Check sheet for the modelled part. Datum: model origin and axes. Units: mm. A direction names the side the tool comes from. Round coordinates to 2 decimals unless told otherwise and drop trailing zeros. Order: outer loops, then holes, each group sorted by start corner. A loop starts at its lowest first (then second) coordinate and runs counter-clockwise, first axis right, second up. Notation, with made-up numbers: M -31.75,81.5 L -11.75,81.5 A16 cw -11.75,91.5 Z; hole C 52,8.5 d8. An arc over 180 degrees is marked long. One line per item, written item: value. Start each with the question number.
(1) Release check for a two-part mould opening along X. For faces 6 (the face through (20, 123, 13)), 7 (the face through (16, 123, -9)), 8 (the face through (-13, 123, -20)) record: released by +X, released by -X, zero draft, split by the parting line, or undercut.
(2) Depth check by flat-ended pin: pin 1 Ø6 at (x, y) = (0, 161.5) entering from +Z; pin 2 Ø3.5 at (y, z) = (152, -2) entering from -X. Enter the tip coordinate at first touch or a pass-through.
(3) Access from +Z, -Z, +X, -X, +Y, -Y to the whole of each face (thin tool, end or side, straight path). Record for faces 1 (the face through (10, 123, 0)), 2 (the face through (-20, 123, -13)), 3 (the face through (-10, 123, 0)), 4 (the face through (-4, 250, 4)), 5 (the face through (-6, 123, -18)).
(4) Cross-section at A-A, the plane z = 0. Enter the section's corners in (x, y).
(5) Thickness scan on L1, parallel to X at y = 71.5, z = 7.5; L2, parallel to Z at x = 18, y = 51; L3, parallel to X at y = 53, z = 0. Record the ranges inside material, lowest first.
(6) Cross-section at B-B, the plane x = 0. Enter the section's corners in (y, z), and give its area (3 significant figures).
from build123d import *

# Parameters (mm, degrees)
SKETCH1_R           = 5
BOSS_EXTRUDE1_DEPTH = 250


with BuildPart() as part:
    # Sketch1 → Boss-Extrude1 (new body)
    with BuildSketch(Plane(origin=(0, 0, 0), x_dir=(1, 0, 0), z_dir=(0, 1, 0))):
        Polygon((-6, 20), (-6, 16), (-11.757359313, 16), (-5.757359313, 10), (5.757359313, 10), (11.757359313, 16), (6, 16), (6, 20), (20, 20), (20, 6), (16, 6), (16, 11.757359313), (10, 5.757359313), (10, -5.757359313), (16, -11.757359313), (16, -6), (20, -6), (20, -20), (6, -20), (6, -16), (11.757359313, -16), (5.757359313, -10), (-5.757359313, -10), (-11.757359313, -16), (-6, -16), (-6, -20), (-20, -20), (-20, -6), (-16, -6), (-16, -11.757359313), (-10, -5.757359313), (-10, 5.757359313), (-16, 11.757359313), (-16, 6), (-20, 6), (-20, 20), align=None)
        with Locations(Location((0, 0, 0), (0, 0, 270))):
            Circle(SKETCH1_R, mode=Mode.SUBTRACT)
    extrude(amount=BOSS_EXTRUDE1_DEPTH)


solid = part.part
Values found:
1. face 6: released by +X
1. face 7: undercut
1. face 8: zero draft
2. pin 1: z = 10
2. pin 2: x = -10
3. face 1: +X, +Y, -Y
3. face 2: +Z, -Z, -X, +Y, -Y
3. face 3: -X, +Y, -Y
3. face 4: +Z, -Z, +X, -X, +Y
3. face 5: -Z, +Y, -Y
4. outline: M -10,0 L -5,0 L -5,250 L -10,250 Z; M 5,0 L 10,0 L 10,250 L 5,250 Z
5. L1: -20 to -16, -11.74 to 11.74, 16 to 20
5. L2: -20 to -6, 6 to 20
5. L3: -10 to -5, 5 to 10
6. outline: M 0,-10 L 250,-10 L 250,-5 L 0,-5 Z; M 0,5 L 250,5 L 250,10 L 0,10 Z
6. area: 2,500 mm^2
